Can you work these out from the model? Positions are in its coordinate system, mm. A direction names the side the tool comes from. Coordinates: 2 decimals unless noted, no trailing zeros. Write each loop counter-clockwise with the first axis right and the second up, starting at its lowest first coordinate (ties: lowest second). Pieces come first, ordered by that corner, then holes. Notation, with made-up numbers: (29, 62.25) -> (77, 62.25) arc R5 cw to (77, 68.25) -> close; hole circle Ø5 at (-19, -27.75). An arc over 180 degrees is marked (long way). Use one line per item in the form item = value.
```python
from build123d import *

# Parameters (mm, degrees)
SKETCH_1_8_R        = 100
SKETCH_1_8_R_2      = 50
SKETCH_1_8_R_3      = 120
BOSS_EXTRUDE1_DEPTH = 45
BOSS_EXTRUDE2_START = -120
SKETCH_1_3_R        = 120
SKETCH_1_3_R_2      = 50
BOSS_EXTRUDE2_DEPTH = 120
BOSS_EXTRUDE3_START = -5
SKETCH_1_4_R        = 100
SKETCH_1_4_R_2      = 50
BOSS_EXTRUDE3_DEPTH = 5
BOSS_EXTRUDE4_START = -120
SKETCH_1_6_R        = 120
SKETCH_1_6_R_2      = 50
SKETCH_1_6_R_3      = 100
BOSS_EXTRUDE4_DEPTH = 45
BOSS_EXTRUDE5_START = -120
SKETCH_1_7_R        = 50
BOSS_EXTRUDE5_DEPTH = 5
BOSS_EXTRUDE6_START = -120
SKETCH_1_8_2_R      = 50
BOSS_EXTRUDE6_DEPTH = 18


with BuildPart() as part:
    # Sketch 1_8 → Boss-Extrude1 (new body)
    # profile 1 of 5: a face of its own
    with BuildSketch(Plane.XY):
        with BuildLine():
            ThreePointArc((13620.744797989, 1922.728345575), (13494.193133773, 1855.229420726), (13430.337526965, 1983.657961365))
            Line((13430.337526965, 1983.657961365), (13198.130204679, 1323.597540284))
            ThreePointArc((13198.130204679, 1323.597540284), (13331.529491927, 1402.061952726), (13431.329633003, 1283.774313052))
            ThreePointArc((13431.329633003, 1283.774313052), (13430.146120976, 1266.962347499), (13426.618929907, 1250.482001337))
            Line((13426.618929907, 1250.482001337), (13620.744797989, 1922.728345575))
        make_face()
    # profile 2 of 5: a face of its own
    with BuildSketch(Plane.XY):
        with Locations((13524.670383902, 1950.471938671)):
            Circle(SKETCH_1_8_R)
        with Locations(Location((13524.670383902, 1950.471938671, 0), (0, 0, 180))):
            Circle(SKETCH_1_8_R_2, mode=Mode.SUBTRACT)
    # profile 3 of 5: a face of its own
    with BuildSketch(Plane.XY):
        with Locations((13311.329633003, 1283.774313052)):
            Circle(SKETCH_1_8_R_3)
        with Locations(Location((13311.329633003, 1283.774313052, 0), (0, 0, 180))):
            Circle(SKETCH_1_8_R_2, mode=Mode.SUBTRACT)
    # profile 4 of 5: a face of its own
    with BuildSketch(Plane.XY):
        with Locations((13705.595707248, 320.324645089)):
            Circle(SKETCH_1_8_R)
        with Locations(Location((13705.595707248, 320.324645089, 0), (0, 0, 180))):
            Circle(SKETCH_1_8_R_2, mode=Mode.SUBTRACT)
    # profile 5 of 5: a face of its own
    with BuildSketch(Plane.XY):
        with BuildLine():
            ThreePointArc((13426.618929907, 1250.482001337), (13318.91585359, 1164.014347884), (13201.162822108, 1236.200436006))
            Line((13201.162822108, 1236.200436006), (13613.790031502, 280.679747551))
            ThreePointArc((13613.790031502, 280.679747551), (13666.552919763, 412.387996893), (13797.912786205, 358.763647846))
            Line((13797.912786205, 358.763647846), (13426.618929907, 1250.482001337))
        make_face()
    extrude(amount=BOSS_EXTRUDE1_DEPTH)

    # 草图1<3> → Boss-Extrude2 (add)
    with BuildSketch(Plane.XY.offset(BOSS_EXTRUDE2_START)):
        with Locations(Location((13311.329633003, 1283.774313052, 0), (0, 0, 160.618277355))):
            Circle(SKETCH_1_3_R)
        with Locations(Location((13311.329633003, 1283.774313052, 0), (0, 0, 180))):
            Circle(SKETCH_1_3_R_2, mode=Mode.SUBTRACT)
    extrude(amount=BOSS_EXTRUDE2_DEPTH)

    # 草图1<4> → Boss-Extrude3 (add)
    # profile 1 of 2: a face of its own
    with BuildSketch(Plane.XY.offset(BOSS_EXTRUDE3_START)):
        with Locations(Location((13524.670383902, 1950.471938671, 0), (0, 0, 160.618277355))):
            Circle(SKETCH_1_4_R)
        with Locations(Location((13524.670383902, 1950.471938671, 0), (0, 0, 180))):
            Circle(SKETCH_1_4_R_2, mode=Mode.SUBTRACT)
    # profile 2 of 2: a face of its own
    with BuildSketch(Plane.XY.offset(BOSS_EXTRUDE3_START)):
        with Locations(Location((13705.595707248, 320.324645089, 0), (0, 0, 203.356373631))):
            Circle(SKETCH_1_4_R)
        with Locations(Location((13705.595707248, 320.324645089, 0), (0, 0, 180))):
            Circle(SKETCH_1_4_R_2, mode=Mode.SUBTRACT)
    extrude(amount=BOSS_EXTRUDE3_DEPTH)



with BuildPart() as body_2:
    # 草图1<6> → Boss-Extrude4 (new body)
    # profile 1 of 5: a face of its own
    with BuildSketch(Plane.XY.offset(BOSS_EXTRUDE4_START)):
        with BuildLine():
            ThreePointArc((13620.744797989, 1922.728345575), (13494.193133773, 1855.229420726), (13430.337526965, 1983.657961365))
            Line((13430.337526965, 1983.657961365), (13198.130204679, 1323.597540284))
            ThreePointArc((13198.130204679, 1323.597540284), (13331.529491927, 1402.061952726), (13431.329633003, 1283.774313052))
            ThreePointArc((13431.329633003, 1283.774313052), (13430.146120976, 1266.962347499), (13426.618929907, 1250.482001337))
            Line((13426.618929907, 1250.482001337), (13620.744797989, 1922.728345575))
        make_face()
    # profile 2 of 5: a face of its own
    with BuildSketch(Plane.XY.offset(BOSS_EXTRUDE4_START)):
        with BuildLine():
            ThreePointArc((13426.618929907, 1250.482001337), (13318.91585359, 1164.014347884), (13201.162822108, 1236.200436006))
            Line((13201.162822108, 1236.200436006), (13613.790031502, 280.679747551))
            ThreePointArc((13613.790031502, 280.679747551), (13666.552919763, 412.387996893), (13797.912786205, 358.763647846))
            Line((13797.912786205, 358.763647846), (13426.618929907, 1250.482001337))
        make_face()
    # profile 3 of 5: a face of its own
    with BuildSketch(Plane.XY.offset(BOSS_EXTRUDE4_START)):
        with Locations(Location((13311.329633003, 1283.774313052, 0), (0, 0, 160.618277355))):
            Circle(SKETCH_1_6_R)
        with Locations(Location((13311.329633003, 1283.774313052, 0), (0, 0, 180))):
            Circle(SKETCH_1_6_R_2, mode=Mode.SUBTRACT)
    # profile 4 of 5: a face of its own
    with BuildSketch(Plane.XY.offset(BOSS_EXTRUDE4_START)):
        with Locations(Location((13705.595707248, 320.324645089, 0), (0, 0, 203.356373631))):
            Circle(SKETCH_1_6_R_3)
        with Locations(Location((13705.595707248, 320.324645089, 0), (0, 0, 180))):
            Circle(SKETCH_1_6_R_2, mode=Mode.SUBTRACT)
    # profile 5 of 5: a face of its own
    with BuildSketch(Plane.XY.offset(BOSS_EXTRUDE4_START)):
        with Locations(Location((13524.670383902, 1950.471938671, 0), (0, 0, 160.618277355))):
            Circle(SKETCH_1_6_R_3)
        with Locations(Location((13524.670383902, 1950.471938671, 0), (0, 0, 180))):
            Circle(SKETCH_1_6_R_2, mode=Mode.SUBTRACT)
    extrude(amount=-BOSS_EXTRUDE4_DEPTH)


with BuildPart() as part_1:
    add(part.part)

    add(body_2.part)  # Boss-Extrude5 merges body 2
    # 草图1<7> → Boss-Extrude5 (add)
    with BuildSketch(Plane.XY.offset(BOSS_EXTRUDE5_START)):
        with BuildLine():
            ThreePointArc((13624.670383902, 1950.471938671), (13541.503599672, 2049.044971732), (13430.337526965, 1983.657961365))
            ThreePointArc((13430.337526965, 1983.657961365), (13494.193133773, 1855.229420726), (13620.744797989, 1922.728345575))
            ThreePointArc((13620.744797989, 1922.728345575), (13623.684123879, 1936.461967377), (13624.670383902, 1950.471938671))
        make_face()
        with Locations(Location((13524.670383902, 1950.471938671, 0), (0, 0, 180))):
            Circle(SKETCH_1_7_R, mode=Mode.SUBTRACT)
    extrude(amount=BOSS_EXTRUDE5_DEPTH)

    # Sketch 1_8 2 → Boss-Extrude6 (add)
    with BuildSketch(Plane.XY.offset(BOSS_EXTRUDE6_START)):
        with BuildLine():
            ThreePointArc((13797.912786205, 358.763647846), (13666.552919763, 412.387996893), (13613.790031502, 280.679747551))
            ThreePointArc((13613.790031502, 280.679747551), (13725.837155139, 222.39465077), (13805.595707248, 320.324645089))
            ThreePointArc((13805.595707248, 320.324645089), (13803.656167924, 339.924289274), (13797.912786205, 358.763647846))
        make_face()
        with Locations(Location((13705.595707248, 320.324645089, 0), (0, 0, 180))):
            Circle(SKETCH_1_8_2_R, mode=Mode.SUBTRACT)
    extrude(amount=BOSS_EXTRUDE6_DEPTH)


solid = part_1.part
```
Q1. Thinking about a two-plate mould opening in X: for faces 1 (the flat face through (13545.5, 1996.3, -115)), 2 (the flat face through (13315.86, 1658.25, 22.18)), 3 (the cylindrical face through (13574.62, 1948.27, 19.65)), which applies, released by +X, released by -X, zero draft, split by the parting line, or undercut?
Return value:
face_1 = zero draft
face_2 = released by -X
face_3 = undercut
Q2. If I drill on line 1 (Z direction, x = 13515.5, y = 993); line 2 (Z direction, x = 13533, y = 1864); line 3 (Y direction, x = 13727.5, z = -145), over which ranges is the centre line in solid material (lowest first)? Write a range as from..to.
Return value:
line_1 = -165..-120, 0..45
line_2 = -165..-115, -5..45
line_3 = 222.75..275.38, 365.27..527.87
Q3. Suppose I cut it at D-D (x = 13691.5). Write out the boundary of the cut face in (y, z), then the cut area to 3 significant figures.
Return value:
outline = (221.32, -165) -> (272.35, -165) -> (272.35, -102) -> (221.32, -102) -> close; (221.32, -5) -> (272.35, -5) -> (272.35, 45) -> (221.32, 45) -> close; (368.3, -165) -> (614.33, -165) -> (614.33, -120) -> (419.33, -120) -> (419.33, -102) -> (368.3, -102) -> close; (368.3, -5) -> (419.33, -5) -> (419.33, 0) -> (614.33, 0) -> (614.33, 45) -> (368.3, 45) -> close
area = 29,100 mm2
Q4. Suppose I cut it at C-C (x = 13515.5). Write out the boundary of the cut face in (y, z).
Return value:
outline = (508.29, -165) -> (1037.02, -165) -> (1037.02, -120) -> (508.29, -120) -> close; (508.29, 0) -> (1037.02, 0) -> (1037.02, 45) -> (508.29, 45) -> close; (1558.27, -165) -> (1901.32, -165) -> (1901.32, -115) -> (1850.89, -115) -> (1850.89, -120) -> (1558.27, -120) -> close; (1558.27, 0) -> (1850.89, 0) -> (1850.89, -5) -> (1901.32, -5) -> (1901.32, 45) -> (1558.27, 45) -> close; (1999.62, -165) -> (2050.05, -165) -> (2050.05, -115) -> (1999.62, -115) -> close; (1999.62, -5) -> (2050.05, -5) -> (2050.05, 45) -> (1999.62, 45) -> close
Q5. For faces 4 (the flat face through (13614.865, 798.381, 22.185)), 5 (the cylindrical face through (13755.547, 318.126, 19.65)), 6 (the flat face through (13659.8, 299.5, -102)), which set-ups out of +Z, -Z, +X, -X, +Y, -Y let a thin tool reach every point of the face, with its end or its side?
Return value:
face_4 = +Z, -Z, +X
face_5 = +Z, -Z
face_6 = +X, -X, +Y, -Y
Q6. Suppose I cut it at A-A (y = 1421.5). Write out the boundary of the cut face in (x, z).
Return value:
outline = (13232.57, -165) -> (13476, -165) -> (13476, -120) -> (13232.57, -120) -> close; (13232.57, 0) -> (13476, 0) -> (13476, 45) -> (13232.57, 45) -> close
Q7. Will these pins go through, and if not, where does the flat tip stop? pin 1 (1 mm diameter, centred on y = 1173.5, z = -47.5, fed in from +X); pin 2 (3 mm diameter, centred on x = 13555.5, z = -120, fed in from -Y).
Return value:
pin_1 = 13359.8
pin_2 = 412.19
Q8. Suppose I cut it at B-B (z = -139). Write out the boundary of the cut face in (x, y), then the cut area to 3 significant figures.
Return value:
outline = (13198.13, 1323.6) arc R120 ccw to (13201.16, 1236.2) -> (13613.79, 280.68) arc R100 ccw to (13797.91, 358.76) -> (13426.62, 1250.48) -> (13620.74, 1922.73) arc R100 ccw to (13430.34, 1983.66) -> close; hole circle Ø100 at (13311.33, 1283.77); hole circle Ø100 at (13524.67, 1950.47); hole circle Ø100 at (13705.6, 320.32)
area = 379,000 mm2
